Geometry check sheet. Reference: the model listing, model coordinates, mm. A direction names the side the tool comes from. Coordinates: 2 decimals unless noted, no trailing zeros. Loops run counter-clockwise (first coordinate to the right, second up) from the corner with the lowest first, then second, coordinate; pieces in that order, holes last. Notation, with made-up numbers: M 26,-16 L 31,-16 A23 ccw 31,14 Z; hole C 44,39 d6. An arc over 180 degrees is marked long. One line per question, with ' | ' between items. Start each with the question number.
from build123d import *

# Parameters (mm, degrees)
STEPPED_BLOCK_BODY_50MM_DEPTH = 25
END_SLOT_PROFILE_30MM_W       = 30
END_SLOT_PROFILE_30MM_H       = 10
END_SLOT_CUT_7_DEEP_DEPTH     = 7
HALF_BORE_CUT_10_DEEP_DEPTH   = 10
CENTRE_BOSS_PROFILE_W         = 15
CENTRE_BOSS_PROFILE_H         = 19.381619709
CENTRE_BOSS_30MM_DEPTH        = 15


with BuildPart() as part:
    # Stepped Block Profile → Stepped Block Body 50mm (new, symmetric)
    with BuildSketch(Plane(origin=(0, 0, 0), x_dir=(0, 0, -1), z_dir=(1, 0, 0))):
        with BuildLine():
            Line((-20, -25), (20, -25))
            Line((20, -25), (20, -45))
            Line((20, -45), (30, -45))
            Line((30, -45), (30, -40))
            Line((30, -40), (55, -40))
            Line((55, -40), (55, -30))
            Line((55, -30), (40, -30))
            Line((40, -30), (40, 20))
            Line((40, 20), (25, 20))
            Line((25, 20), (15, 30))
            Line((15, 30), (7.5, 30))
            Line((7.5, 30), (7.5, 10.618380291))
            ThreePointArc((7.5, 10.618380291), (0, -13), (-7.5, 10.618380291))
            Line((-7.5, 10.618380291), (-7.5, 30))
            Line((-7.5, 30), (-15, 30))
            Line((-15, 30), (-25, 20))
            Line((-25, 20), (-40, 20))
            Line((-40, 20), (-40, -30))
            Line((-40, -30), (-55, -30))
            Line((-55, -30), (-55, -40))
            Line((-55, -40), (-30, -40))
            Line((-30, -40), (-30, -45))
            Line((-30, -45), (-20, -45))
            Line((-20, -45), (-20, -25))
        make_face()
    extrude(amount=STEPPED_BLOCK_BODY_50MM_DEPTH, both=True)

    # End Slot Profile 30mm → End Slot Cut 7 Deep (cut)
    with BuildSketch(Plane.XY.offset(55)):
        with Locations((0, -35)):
            Rectangle(END_SLOT_PROFILE_30MM_W, END_SLOT_PROFILE_30MM_H)
    end_slot_cut_7_deep = extrude(amount=-END_SLOT_CUT_7_DEEP_DEPTH, mode=Mode.SUBTRACT)

    # Half Bore Profile → Half Bore Cut 10 Deep (cut)
    with BuildSketch(Plane.XY.offset(40)):
        with BuildLine():
            Line((-17, 20), (17, 20))
            ThreePointArc((17, 20), (0, 3), (-17, 20))
        make_face()
    half_bore_cut_10_deep = extrude(amount=-HALF_BORE_CUT_10_DEEP_DEPTH, mode=Mode.SUBTRACT)

    # End Slot and Bore Mirror: End Slot Cut 7 Deep, Half Bore Cut 10 Deep across plane
    add(end_slot_cut_7_deep.mirror(Plane.XY), mode=Mode.SUBTRACT)
    add(half_bore_cut_10_deep.mirror(Plane.XY), mode=Mode.SUBTRACT)

    # Centre Boss Profile → Centre Boss 30mm (add, symmetric)
    with BuildSketch(Plane(origin=(0, 0, 0), x_dir=(0, 0, -1), z_dir=(1, 0, 0))):
        with Locations((0, 20.309190146)):
            Rectangle(CENTRE_BOSS_PROFILE_W, CENTRE_BOSS_PROFILE_H)
    extrude(amount=CENTRE_BOSS_30MM_DEPTH, both=True)


solid = part.part
1. Sectioned sample at A-A (y = 0). Record the cut outline in (x, z), and give its area (3 significant figures).
2. Depth check by flat-ended pin: pin 1 Ø7.5 at (x, z) = (-3.5, -31.5) entering from +Y; pin 2 Ø15 at (x, y) = (-3.5, 7) entering from -Z; pin 3 Ø1.5 at (x, y) = (-9.5, -43.5) entering from +Z. Enter the tip coordinate at first touch or a pass-through.
3. Draft check along Y on faces 5 (the flat face through (0, 20, -29)), 6 (the flat face through (-25, -15, 1)), 7 (the flat face through (0, 10.618, 0)). Enter one of: +Y half, -Y half, draft (parallel to the pull), parting line (faces both ways), or undercut.
4. Tool access check on faces 1 (the flat face through (0, -42, 30)), 2 (the flat face through (20, 20, 7.5)), 3 (the flat face through (0, -11, -40)), 4 (the flat face through (0, -35, 48)). Record the directions out of +Z, -Z, +X, -X, +Y, -Y that give a thin tool (end or side, any length) a straight path to the whole face; none if there is none.
5. Sectioned sample at C-C (z = -5). Record the cut outline in (x, y), and give its area (3 significant figures).
6. Sectioned sample at D-D (x = 19.5). Record the cut outline in (y, z), and give its area (3 significant figures).
7. Thickness scan on line 1 (Z direction, x = 4, y = 0); line 2 (Y direction, x = 4, z = 0); line 3 (X direction, y = 13.5, z = 2.5). Record the ranges inside material, lowest first.
8. Sectioned sample at B-B (x = 0). Record the cut outline in (y, z).
Result:
1) outline: M -25,-40 L 25,-40 L 25,-13 L -25,-13 Z; M -25,13 L 25,13 L 25,40 L -25,40 Z | area: 2,700 mm2
2) pin 1: stops at y = 20 | pin 2: stops at z = -40 | pin 3: stops at z = 30
3) face 5: +Y half | face 6: draft | face 7: undercut
4) face 1: +Z, +X, -X, -Y | face 2: +X, +Y | face 3: -Z, +X, -X, +Y | face 4: +Z, +Y, -Y
5) outline: M -25,-25 L 25,-25 L 25,-12 L -25,-12 Z; M -15,10.62 L 15,10.62 L 15,30 L -15,30 Z | area: 1,230 mm2
6) outline: M -45,-30 L -40,-30 L -40,-55 L -30,-55 L -30,-40 L 20,-40 L 20,-25 L 30,-15 L 30,-7.5 L 10.62,-7.5 A13 cw long 10.62,7.5 L 30,7.5 L 30,15 L 20,25 L 20,40 L -30,40 L -30,55 L -40,55 L -40,30 L -45,30 L -45,20 L -25,20 L -25,-20 L -45,-20 Z | area: 4,200 mm2
7) line 1: z = -40 to -13, 13 to 40 | line 2: y = -25 to -13, 10.62 to 30 | line 3: x = -15 to 15
8) outline: M -45,-30 L -40,-30 L -40,-48 L -30,-48 L -30,-40 L 3,-40 L 3,-30 L 20,-30 L 20,-25 L 30,-15 L 30,15 L 20,25 L 20,30 L 3,30 L 3,40 L -30,40 L -30,48 L -40,48 L -40,30 L -45,30 L -45,20 L -25,20 L -25,-20 L -45,-20 Z; hole M 10.62,-7.5 L 10.62,7.5 A13 ccw long Z
